```python
from build123d import *

# Parameters (mm, degrees)
STEM_PROFILE_36_R           = 18
STEM_36X44_DEPTH            = 44
BASE_PLATE_PROFILE_W        = 88
BASE_PLATE_PROFILE_H        = 36
BASE_PLATE_88X36X6_DEPTH    = 6
LUG_PROFILE_WITH_PIN_HOLE_R = 7.5
LUG_6MM_DEPTH               = 6


with BuildPart() as part:
    # Stem Profile Ø36 → Stem Ø36x44 (new body)
    with BuildSketch(Plane(origin=(0, 0, 0), x_dir=(1, 0, 0), z_dir=(0, 1, 0))):
        with Locations(Location((0, 0, 0), (0, 0, 270))):
            Circle(STEM_PROFILE_36_R)
    extrude(amount=STEM_36X44_DEPTH)

    # Base Plate Profile → Base Plate 88x36x6 (add)
    with BuildSketch(Plane(origin=(0, 44, 0), x_dir=(1, 0, 0), z_dir=(0, 1, 0))):
        Rectangle(BASE_PLATE_PROFILE_W, BASE_PLATE_PROFILE_H)
    extrude(amount=BASE_PLATE_88X36X6_DEPTH)

    # Lug Profile with Pin Hole → Lug 6mm (add)
    with BuildSketch(Plane(origin=(44, 0, 0), x_dir=(0, 0, -1), z_dir=(1, 0, 0))):
        with BuildLine():
            Line((-18, 44), (18, 44))
            Line((18, 44), (18, 92))
            ThreePointArc((18, 92), (0, 110), (-18, 92))
            Line((-18, 92), (-18, 44))
        make_face()
        with Locations((0, 92)):
            Circle(LUG_PROFILE_WITH_PIN_HOLE_R, mode=Mode.SUBTRACT)
    lug_6mm = extrude(amount=LUG_6MM_DEPTH)

    # Lug Mirror: Lug 6mm across plane
    add(lug_6mm.mirror(Plane(origin=(0, 0, 0), x_dir=(0, 0, 1), z_dir=(1, 0, 0))))


solid = part.part
```
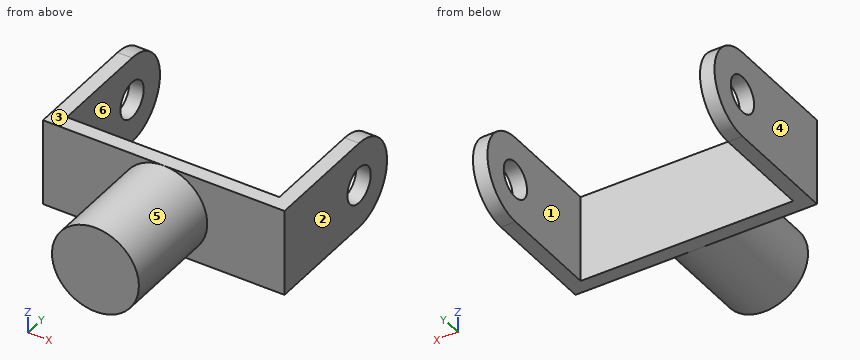
Can you work these out from the model? Positions are in its coordinate system, mm. Face numbers are marked on the shaded views. A direction names the side the tool comes from. Coordinates: 2 decimals unless noted, no trailing zeros. Loops run counter-clockwise (first coordinate to the right, second up) from the corner with the lowest first, then second, coordinate; pieces in that order, holes last. Notation, with made-up numbers: (34, 30.5) - (49, 30.5) arc R19 ccw to (49, 57.5) - close; hole circle Ø5 at (61, 29). An arc over 180 degrees is marked (long way). Answer as CSV lines item,"result". Start each with the question number.
1) Thinking about a two-plate mould opening in X: for the marked faces 1, 2 and 3, which applies, pulls with the +X half, pulls with the -X half, needs draft (parallel to the pull), parting line crosses it, or undercut?
2) Suppose I cut it at A-A (z = 0). Please give me the cut outline in (x, y).
3) Which directions (+Z, -Z, +X, -X, +Y, -Y) give clear straight access to the entire face, cutting with the end or side of a thin tool? Please do the marked faces 4, 5 and 6.
4) Suppose I cut it at D-D (z = -13). Please give me the cut outline in (x, y).
5) Suppose I cut it at B-B (y = 97.5). Please give me the cut outline in (x, z).
6) Suppose I cut it at C-C (x = 12). Please give me the cut outline in (y, z), plus the area to 3 significant figures.
7) For pin 1 (8 mm diameter, centred on x = 31, z = 11.5, fed in from +Y), with a flat end and sliding along its axis, tell me the tip position at first contact or that it passes through.
8) I need wall thicknesses on line 1 (Y direction, x = -47, z = 0); line 2 (X direction, y = 83, z = -7); line 3 (Y direction, x = -27, z = 16). Which ranges of each line are inside material? Lowest first, please. Write a range as from..to.
Check result:
1,face 1,"undercut"
1,face 2,"pulls with the +X half"
1,face 3,"needs draft"
2,outline,"(-50, 44) - (-18, 44) - (-18, 0) - (18, 0) - (18, 44) - (50, 44) - (50, 84.5) - (44, 84.5) - (44, 50) - (-44, 50) - (-44, 84.5) - (-50, 84.5) - close; (-50, 99.5) - (-44, 99.5) - (-44, 110) - (-50, 110) - close; (44, 99.5) - (50, 99.5) - (50, 110) - (44, 110) - close"
3,face 4,"+Z, -Z, -X, +Y, -Y"
3,face 5,"-Y"
3,face 6,"+Z, -Z, +Y"
4,outline,"(-50, 44) - (-12.45, 44) - (-12.45, 0) - (12.45, 0) - (12.45, 44) - (50, 44) - (50, 104.45) - (44, 104.45) - (44, 50) - (-44, 50) - (-44, 104.45) - (-50, 104.45) - close"
5,outline,"(-50, -17.14) - (-44, -17.14) - (-44, -5.1) - (-50, -5.1) - close; (-50, 5.1) - (-44, 5.1) - (-44, 17.14) - (-50, 17.14) - close; (44, -17.14) - (50, -17.14) - (50, -5.1) - (44, -5.1) - close; (44, 5.1) - (50, 5.1) - (50, 17.14) - (44, 17.14) - close"
6,outline,"(0, -13.42) - (44, -13.42) - (44, -18) - (50, -18) - (50, 18) - (44, 18) - (44, 13.42) - (0, 13.42) - close"
6,area,"1,400 mm²"
7,pin 1,"stops at y = 50"
8,line 1,"y = 44..84.5, 99.5..110"
8,line 2,"x = -50..-44, 44..50"
8,line 3,"y = 44..50"
